```python
from build123d import *

# Parameters (mm, degrees)
BOSS_EXTRUDE1_DEPTH            = 30
SKETCH2_W                      = 8
SKETCH2_H                      = 30
BOSS_EXTRUDE2_DEPTH            = 8
SKETCH3_W                      = 8
SKETCH3_H                      = 16
BOSS_EXTRUDE3_DEPTH            = 15
SKETCH4_W                      = 45
SKETCH4_H                      = 16
BOSS_EXTRUDE4_DEPTH            = 195
SKETCH5_W                      = 45
SKETCH5_H                      = 16
BOSS_EXTRUDE5_DEPTH            = 347
SKETCH6_W                      = 347
SKETCH6_H                      = 30
CUT_EXTRUDE1_DEPTH             = 3
SKETCH7_W                      = 30
SKETCH7_H                      = 5
CUT_EXTRUDE2_DEPTH             = 150
SKETCH8_W                      = 30
SKETCH8_H                      = 13
CUT_EXTRUDE3_DEPTH             = 20
SKETCH9_W                      = 150
SKETCH9_H                      = 30
CUT_EXTRUDE4_DEPTH             = 5
SKETCH10_W                     = 550
SKETCH10_H                     = 16
BOSS_EXTRUDE6_DEPTH            = 355
SKETCH11_W                     = 450
SKETCH11_H                     = 340
CUT_EXTRUDE5_DEPTH             = 681.261714342
F_10_0_10_DIAMETER_HOLE1_D     = 10
F_10_0_10_DIAMETER_HOLE1_DEPTH = 20
F_10_0_10_DIAMETER_HOLE2_D     = 10
F_10_0_10_DIAMETER_HOLE2_DEPTH = 15
F_10_0_10_DIAMETER_HOLE3_D     = 10
F_10_0_10_DIAMETER_HOLE3_DEPTH = 355


with BuildPart() as part:
    # Sketch1 → Boss-Extrude1 (new body)
    with BuildSketch(Plane(origin=(0, 0, -45), x_dir=(-1, 0, 0), z_dir=(0, 0, -1))):
        Polygon((-355, -8), (-347, -8), (-355, 0), align=None)
    extrude(amount=-BOSS_EXTRUDE1_DEPTH)

    # Sketch2 → Boss-Extrude2 (add)
    with BuildSketch(Plane.XZ.offset(8)):
        with Locations((351, -30)):
            Rectangle(SKETCH2_W, SKETCH2_H)
    extrude(amount=BOSS_EXTRUDE2_DEPTH)

    # Sketch3 → Boss-Extrude3 (add)
    with BuildSketch(Plane.XY.offset(-15)):
        with Locations((351, -8)):
            Rectangle(SKETCH3_W, SKETCH3_H)
    extrude(amount=BOSS_EXTRUDE3_DEPTH)

    # Sketch4 → Boss-Extrude4 (add)
    with BuildSketch(Plane(origin=(355, 0, 0), x_dir=(0, 0, -1), z_dir=(1, 0, 0))):
        with Locations((22.5, -8)):
            Rectangle(SKETCH4_W, SKETCH4_H)
    extrude(amount=BOSS_EXTRUDE4_DEPTH)

    # Sketch5 → Boss-Extrude5 (add)
    with BuildSketch(Plane.ZY.offset(-347)):
        with Locations((-22.5, -8)):
            Rectangle(SKETCH5_W, SKETCH5_H)
    extrude(amount=BOSS_EXTRUDE5_DEPTH)

    # Sketch6 → Cut-Extrude1 (cut)
    with BuildSketch(Plane(origin=(0, 0, 0), x_dir=(-1, 0, 0), z_dir=(0, 1, 0))):
        with Locations((-173.5, -30)):
            Rectangle(SKETCH6_W, SKETCH6_H)
    extrude(amount=-CUT_EXTRUDE1_DEPTH, mode=Mode.SUBTRACT)

    # Sketch7 → Cut-Extrude2 (cut)
    with BuildSketch(Plane(origin=(347, 0, 0), x_dir=(0, 0, -1), z_dir=(1, 0, 0))):
        with Locations((30, -5.5)):
            Rectangle(SKETCH7_W, SKETCH7_H)
    extrude(amount=-CUT_EXTRUDE2_DEPTH, mode=Mode.SUBTRACT)

    # Sketch8 → Cut-Extrude3 (cut)
    with BuildSketch(Plane(origin=(197, 0, 0), x_dir=(0, 0, -1), z_dir=(1, 0, 0))):
        with Locations((30, -9.5)):
            Rectangle(SKETCH8_W, SKETCH8_H)
    extrude(amount=-CUT_EXTRUDE3_DEPTH, mode=Mode.SUBTRACT)

    # Sketch9 → Cut-Extrude4 (cut)
    with BuildSketch(Plane(origin=(0, -8, 0), x_dir=(-1, 0, 0), z_dir=(0, 1, 0))):
        with Locations((-272, -30)):
            Rectangle(SKETCH9_W, SKETCH9_H)
    extrude(amount=-CUT_EXTRUDE4_DEPTH, mode=Mode.SUBTRACT)

    # Sketch10 → Boss-Extrude6 (add)
    with BuildSketch(Plane(origin=(0, 0, -45), x_dir=(-1, 0, 0), z_dir=(0, 0, -1))):
        with Locations((-275, -8)):
            Rectangle(SKETCH10_W, SKETCH10_H)
    extrude(amount=BOSS_EXTRUDE6_DEPTH)

    # Sketch11 → Cut-Extrude5 (cut, through all)
    with BuildSketch(Plane(origin=(0, 0, 0), x_dir=(-1, 0, 0), z_dir=(0, 1, 0))):
        with Locations((-275, -230)):
            Rectangle(SKETCH11_W, SKETCH11_H)
    extrude(amount=-CUT_EXTRUDE5_DEPTH, mode=Mode.SUBTRACT)

    # Ø10.0 (10) Diameter Hole1
    with Locations(Plane.XY):
        with Locations((437, -8)):
            Hole(F_10_0_10_DIAMETER_HOLE1_D / 2, depth=F_10_0_10_DIAMETER_HOLE1_DEPTH)

    # Ø10.0 (10) Diameter Hole2
    with Locations(Plane.XY):
        with Locations((187, -8)):
            Hole(F_10_0_10_DIAMETER_HOLE2_D / 2, depth=F_10_0_10_DIAMETER_HOLE2_DEPTH)

    # Ø10.0 (10) Diameter Hole3
    with Locations(Plane.XY.offset(-45)):
        with Locations((187, -8)):
            Hole(F_10_0_10_DIAMETER_HOLE3_D / 2, depth=F_10_0_10_DIAMETER_HOLE3_DEPTH)


solid = part.part
```
Build history of the part. All positions in model axes, mm. A direction names the side the tool comes from. Give positions to 0.01 mm unless a question says otherwise; leave off trailing zeros. Loops run counter-clockwise (first coordinate to the right, second up) from the corner with the lowest first, then second, coordinate; pieces in that order, holes last. Notation, with made-up numbers: (40, -5) -> (99, -5) arc R34 ccw to (99, 26) -> close; hole circle Ø11 at (-40, 24.5). An arc over 180 degrees is marked (long way). One line per question, with ' | ' between items. Start each with the question number.
1) 3-axis set-ups, long thin cutter, end or side, ignore diameter. For faces 5 (the flat face through (50, -8, -232)), 6 (the flat face through (214, -4, -15)), 7 (the flat face through (177, -9, -30)): which of +Z, -Z, +X, -X, +Y, -Y reach the whole face in a straight line?
2) Cut at C-C (x = 393). Give the cut face in (y, z), plus the area to 3 significant figures.
3) Pin check, flat tips, straight feed: pin 1 (24 mm diameter, centred on x = 282, z = -33.5, fed in from +Y); pin 2 (8 mm diameter, centred on x = 370.5, y = -9, fed in from -Z); pin 3 (3 mm diameter, centred on x = 438.5, y = -9, fed in from +Z). Stop position of each tip, or through.
4) Cut at A-A (z = -375). Give the cut face in (x, y), plus the area to 3 significant figures.
5) Probe L1, parallel to X at y = -11.25, z = -87.5; L2, parallel to Z at x = 296.5, y = -10.75; L3, parallel to Z at x = 173, y = -8. List the from-to ranges inside material, lowest first.
6) Cut at B-B (x = 86). Give the cut face in (y, z), plus the area to 3 significant figures.
7) Two-plate mould, pull along X, no slides. Class faces 1 (the flat face through (273, -13, -30)), 2 (the flat face through (550, -8, -197)), 3 (the flat face through (317, 0, -51)), 4 (the flat face through (278, -8, -60)): released by +X, released by -X, zero draft, split by the parting line, or undercut.
Return value:
1) face 5: -Z, +Y, -Y | face 6: +Y | face 7: +Y, -Y
2) outline: (-16, -60) -> (0, -60) -> (0, 0) -> (-16, 0) -> close | area: 960 mm^2
3) pin 1: y = 0 | pin 2: z = -60 | pin 3: z = -20
4) outline: (0, -16) -> (50, -16) -> (50, 0) -> (0, 0) -> close; (500, -16) -> (550, -16) -> (550, 0) -> (500, 0) -> close | area: 1,600 mm^2
5) L1: 0 to 50, 500 to 550 | L2: -60 to -45, -15 to 0 | L3: -60 to 0
6) outline: (-16, -60) -> (0, -60) -> (0, -45) -> (-3, -45) -> (-3, -15) -> (0, -15) -> (0, 0) -> (-16, 0) -> close | area: 870 mm^2
7) face 1: undercut | face 2: released by +X | face 3: zero draft | face 4: undercut
